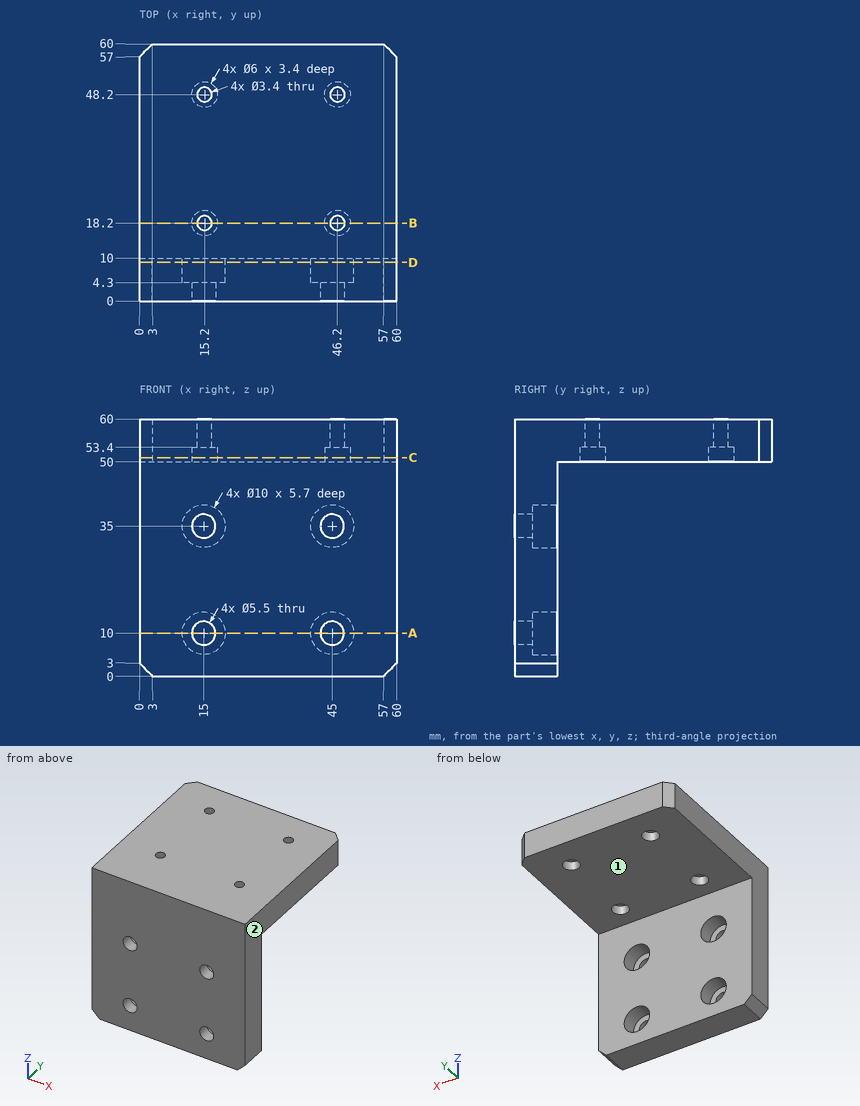
Geometry: see drawing. Coordinates: mm, zero at the bounding-box minimum. A direction names the side the tool comes from. Give positions to 0.01 mm unless a question says otherwise; leave off trailing zeros. Loops run counter-clockwise (first coordinate to the right, second up) from the corner with the lowest first, then second, coordinate; pieces in that order, holes last. Notation, with made-up numbers: (-26, 8) - (25, 8) arc R14 ccw to (25, 20) - close; hole circle Ø3 at (-33.75, 89.5). An arc over 180 degrees is marked (long way). One line per question, with ' | ' between items. Start each with the question number.
(1) Section query B-B on y = 18.2. Return loops of the section in (x, z), then the cut area to 3 significant figures.
(2) Reachability of the marked faces 1 and 2 from +Z, -Z, +X, -X, +Y, -Y: full face, straight path, thin tool, end or side. Return the list, or none.
(3) Section query D-D on y = 9. Return loops of the section in (x, z), then the cut area to 3 significant figures.
(4) Section query C-C on z = 51. Return loops of the section in (x, y), then the cut area to 3 significant figures.
(5) Ray query, line 1 (Z direction, x = 15, y = 3.2); line 2 (X direction, y = 2, z = 35); line 3 (X direction, y = 48, z = 56). Return the intervals inside material, ascending. Write a range as from..to.
(6) Contact query for flat-ended pins moving along their axis: pin 1 (4.5 mm diameter, centred on x = 46.2, y = 48.2, fed in from -Z); pin 2 (3 mm diameter, centred on x = 38, z = 21, fed in from +Y); pin 3 (3 mm diameter, centred on x = 15, z = 7.5, fed in from +Y); pin 4 (13 mm diameter, centred on x = 45, z = 35, fed in from -Y). Output: stop coordinate, or through.
(7) Section query A-A on z = 10. Return loops of the section in (x, y), then the cut area to 3 significant figures.
The answers:
1) outline: (0, 50) - (12.2, 50) - (12.2, 53.4) - (13.5, 53.4) - (13.5, 60) - (0, 60) - close; (16.9, 53.4) - (18.2, 53.4) - (18.2, 50) - (43.2, 50) - (43.2, 53.4) - (44.5, 53.4) - (44.5, 60) - (16.9, 60) - close; (47.9, 53.4) - (49.2, 53.4) - (49.2, 50) - (60, 50) - (60, 60) - (47.9, 60) - close | area: 514 mm2
2) face 1: -Z, +X, -X, +Y | face 2: +Z, -Z, +X, +Y, -Y
3) outline: (0, 3) - (3, 0) - (57, 0) - (60, 3) - (60, 60) - (0, 60) - close; hole circle Ø10 at (15, 10); hole circle Ø10 at (15, 35); hole circle Ø10 at (45, 10); hole circle Ø10 at (45, 35) | area: 3,280 mm2
4) outline: (0, 0) - (60, 0) - (60, 57) - (57, 60) - (3, 60) - (0, 57) - close; hole circle Ø6 at (15.2, 18.2); hole circle Ø6 at (15.2, 48.2); hole circle Ø6 at (46.2, 18.2); hole circle Ø6 at (46.2, 48.2) | area: 3,480 mm2
5) line 1: 0..7.25, 12.75..32.25, 37.75..60 | line 2: 0..12.25, 17.75..42.25, 47.75..60 | line 3: 0..13.51, 16.89..44.51, 47.89..60
6) pin 1: z = 53.4 | pin 2: y = 10 | pin 3: y = 4.3 | pin 4: y = 0
7) outline: (0, 0) - (12.25, 0) - (12.25, 4.3) - (10, 4.3) - (10, 10) - (0, 10) - close; (17.75, 0) - (42.25, 0) - (42.25, 4.3) - (40, 4.3) - (40, 10) - (20, 10) - (20, 4.3) - (17.75, 4.3) - close; (47.75, 0) - (60, 0) - (60, 10) - (50, 10) - (50, 4.3) - (47.75, 4.3) - close | area: 439 mm2
